The listing builds one solid part. Answer for the finished solid, in the listing's coordinates (mm). Face numbers are marked on the shaded views. A direction names the side the tool comes from. Give positions to 0.01 mm unless a question says otherwise; leave off trailing zeros. Write each loop counter-clockwise with the first axis right and the second up, starting at its lowest first coordinate (ties: lowest second). Pieces come first, ordered by that corner, then holes. Notation, with made-up numbers: M 40.5,5 L 93.5,5 A25 cw 93.5,38 Z; hole C -28,-6.5 d4. An arc over 180 degrees is marked long. Answer as a JSON object with one key per item and string values.
```python
from build123d import *

# Parameters (mm, degrees)
SKETCH_1_R          = 5.25
EXTRUDE_1_DEPTH     = 3.2
SKETCH_2_R          = 27
CUT_EXTRUDE_1_DEPTH = 1.5
SKETCH_3_R          = 13.5
EXTRUDE_2_DEPTH     = 1


with BuildPart() as part:
    # 草图1 → 凸台-拉伸1 (new body)
    with BuildSketch(Plane(origin=(0, 0, 0), x_dir=(1, 0, 0), z_dir=(0, 1, 0))):
        with BuildLine():
            Line((-35.5, -45), (35.5, -45))
            ThreePointArc((35.5, -45), (42.217514421, -42.217514421), (45, -35.5))
            Line((45, -35.5), (45, 35.5))
            ThreePointArc((45, 35.5), (42.217514421, 42.217514421), (35.5, 45))
            Line((35.5, 45), (-35.5, 45))
            ThreePointArc((-35.5, 45), (-42.217514421, 42.217514421), (-45, 35.5))
            Line((-45, 35.5), (-45, -35.5))
            ThreePointArc((-45, -35.5), (-42.217514421, -42.217514421), (-35.5, -45))
        make_face()
        with Locations(Location((35.5, -35.5, 0), (0, 0, 270))):
            Circle(SKETCH_1_R, mode=Mode.SUBTRACT)
        with Locations(Location((35.5, 35.5, 0), (0, 0, 270))):
            Circle(SKETCH_1_R, mode=Mode.SUBTRACT)
        with Locations(Location((-35.5, -35.5, 0), (0, 0, 270))):
            Circle(SKETCH_1_R, mode=Mode.SUBTRACT)
        with Locations(Location((-35.5, 35.5, 0), (0, 0, 270))):
            Circle(SKETCH_1_R, mode=Mode.SUBTRACT)
    extrude(amount=-EXTRUDE_1_DEPTH)

    # 草图2 → 切除-拉伸1 (cut)
    with BuildSketch(Plane(origin=(0, 0, 0), x_dir=(1, 0, 0), z_dir=(0, 1, 0))):
        with Locations(Location((0, 0, 0), (0, 0, 270))):
            Circle(SKETCH_2_R)
    extrude(amount=-CUT_EXTRUDE_1_DEPTH, mode=Mode.SUBTRACT)

    # 草图3 → 凸台-拉伸2 (add)
    with BuildSketch(Plane(origin=(0, -1.5, 0), x_dir=(1, 0, 0), z_dir=(0, 1, 0))):
        with Locations(Location((0, 0, 0), (0, 0, 270))):
            Circle(SKETCH_3_R)
    extrude(amount=EXTRUDE_2_DEPTH)

    # 草图4 → 旋转1 (revolve)
    with BuildSketch(Plane(origin=(0, 0, 0), x_dir=(0, 0, -1), z_dir=(1, 0, 0))):
        with BuildLine():
            Line((0, -14.2), (-29.255663301, -14.2))
            ThreePointArc((-29.255663301, -14.2), (-31.091107897, -13.621286542), (-32.262679687, -12.094464459))
            Line((-32.262679687, -12.094464459), (-35.5, -3.2))
            Line((-35.5, -3.2), (0, -3.2))
            Line((0, -3.2), (0, -14.2))
        make_face()
    revolve(axis=Axis((0, -3.2, 0), (0, -1, 0)))


solid = part.part
```
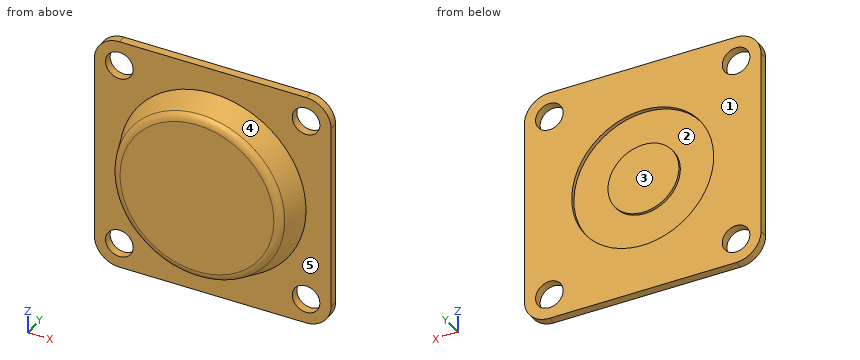
1. The mould has two halves that part along Z. Classify the marked faces 3, 4 and 5: released by +Z, released by -Z, zero draft, split by the parting line, or undercut.
Verdict:
{"face 3": "undercut", "face 4": "split by the parting line", "face 5": "zero draft"}
2. A cutting plane is placed at C-C, the plane y = -9.25. Give the vertices of the cut face in (x, z), plus the area to 3 significant figures.
Verdict:
{"outline": "C 0,0 d66.6", "area": "3,480 mm2"}
3. A cutting plane is placed at B-B, the plane x = -38. Give the vertices of the cut face in (y, z), plus the area to 3 significant figures.
Verdict:
{"outline": "M -3.2,-44.67 L 0,-44.67 L 0,-40.12 L -3.2,-40.12 Z; M -3.2,-30.88 L 0,-30.88 L 0,30.88 L -3.2,30.88 Z; M -3.2,40.12 L 0,40.12 L 0,44.67 L -3.2,44.67 Z", "area": "227 mm2"}
4. Flat-ended cylindrical pins translate along their axes: pin 1 (21.5 mm diameter, centred on x = 6, z = -1.5, fed in from +Y); pin 2 (8 mm diameter, centred on x = 35.5, z = 25.5, fed in from -Y); pin 3 (5 mm diameter, centred on x = 17, z = -6, fed in from +Y). Find the tip coordinate at first contact, or state that the pin passes through.
Verdict:
{"pin 1": "stops at y = -0.5", "pin 2": "stops at y = -3.2", "pin 3": "stops at y = -1.5"}
5. For the marked faces 1 and 2, determine the directions among +Z, -Z, +X, -X, +Y, -Y from which every point of the face is accessible in a straight line to the end or side of a thin tool.
Verdict:
{"face 1": "+Z, -Z, +X, -X, +Y", "face 2": "+Y"}
6. Consider line 1 along X through (y, z) = (-1.5, 35.5); line 2 along Y through (x, z) = (11.5, 12.5); line 3 along Y through (x, z) = (12, -1.5). Determine where each line is inside the solid, lowest interval first.
Verdict:
{"line 1": "x = -45 to -40.75, -30.25 to 30.25, 40.75 to 45", "line 2": "y = -14.2 to -1.5", "line 3": "y = -14.2 to -0.5"}
7. A cutting plane is placed at A-A, the plane z = 0. Give the vertices of the cut face in (x, y).
Verdict:
{"outline": "M -45,-3.2 L -35.5,-3.2 L -32.26,-12.09 A3.2 ccw -29.26,-14.2 L 29.26,-14.2 A3.2 ccw 32.26,-12.09 L 35.5,-3.2 L 45,-3.2 L 45,0 L 27,0 L 27,-1.5 L 13.5,-1.5 L 13.5,-0.5 L -13.5,-0.5 L -13.5,-1.5 L -27,-1.5 L -27,0 L -45,0 Z"}
